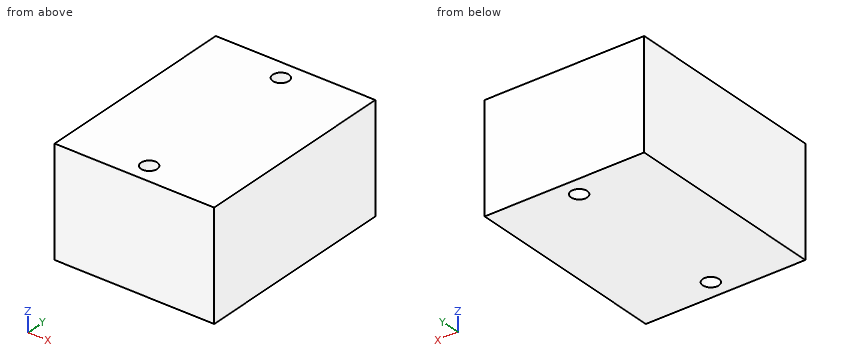
```python
from build123d import *

# Parameters (mm, degrees)
SKETCH_1_W      = 44.5
SKETCH_1_H      = 58
SKETCH_1_R      = 2.25
EXTRUDE_1_DEPTH = 30


with BuildPart() as part:
    # 草图1 → 凸台-拉伸1 (new body)
    with BuildSketch(Plane.XY):
        Rectangle(SKETCH_1_W, SKETCH_1_H)
        with Locations((0, 23.7)):
            Circle(SKETCH_1_R, mode=Mode.SUBTRACT)
        with Locations((0, -23.7)):
            Circle(SKETCH_1_R, mode=Mode.SUBTRACT)
    extrude(amount=EXTRUDE_1_DEPTH)


solid = part.part
```
The listing builds one solid part. Answer for the finished solid, in the listing's coordinates (mm). Give positions to 0.01 mm unless a question says otherwise; leave off trailing zeros. Order: outer loops, then holes, each group sorted by start corner. A loop starts at its lowest first (then second) coordinate and runs counter-clockwise, first axis right, second up. Notation, with made-up numbers: (-4, -23.5) -> (17, -23.5) arc R20 ccw to (17, -11.5) -> close; hole circle Ø4 at (-14.5, 69.5). An arc over 180 degrees is marked (long way). Answer as CSV lines item,"result". Start each with the question number.
Q1. Find the intervals of material crossed by L1, parallel to X at y = -23.5, z = 28.5; L2, parallel to Y at x = -2, z = 8; L3, parallel to X at y = -22, z = 12.25, in increasing order.
Q2. A cutting plane is placed at A-A (x = 0). Determine the outline of the cut face in (y, z), then the cut area to 3 significant figures.
Q3. A cutting plane is placed at B-B (y = 23.7). Determine the outline of the cut face in (x, z).
Results found:
1,L1,"-22.25 to -2.24, 2.24 to 22.25"
1,L2,"-29 to -24.73, -22.67 to 22.67, 24.73 to 29"
1,L3,"-22.25 to -1.47, 1.47 to 22.25"
2,outline,"(-29, 0) -> (-25.95, 0) -> (-25.95, 30) -> (-29, 30) -> close; (-21.45, 0) -> (21.45, 0) -> (21.45, 30) -> (-21.45, 30) -> close; (25.95, 0) -> (29, 0) -> (29, 30) -> (25.95, 30) -> close"
2,area,"1,470 mm2"
3,outline,"(-22.25, 0) -> (-2.25, 0) -> (-2.25, 30) -> (-22.25, 30) -> close; (2.25, 0) -> (22.25, 0) -> (22.25, 30) -> (2.25, 30) -> close"
